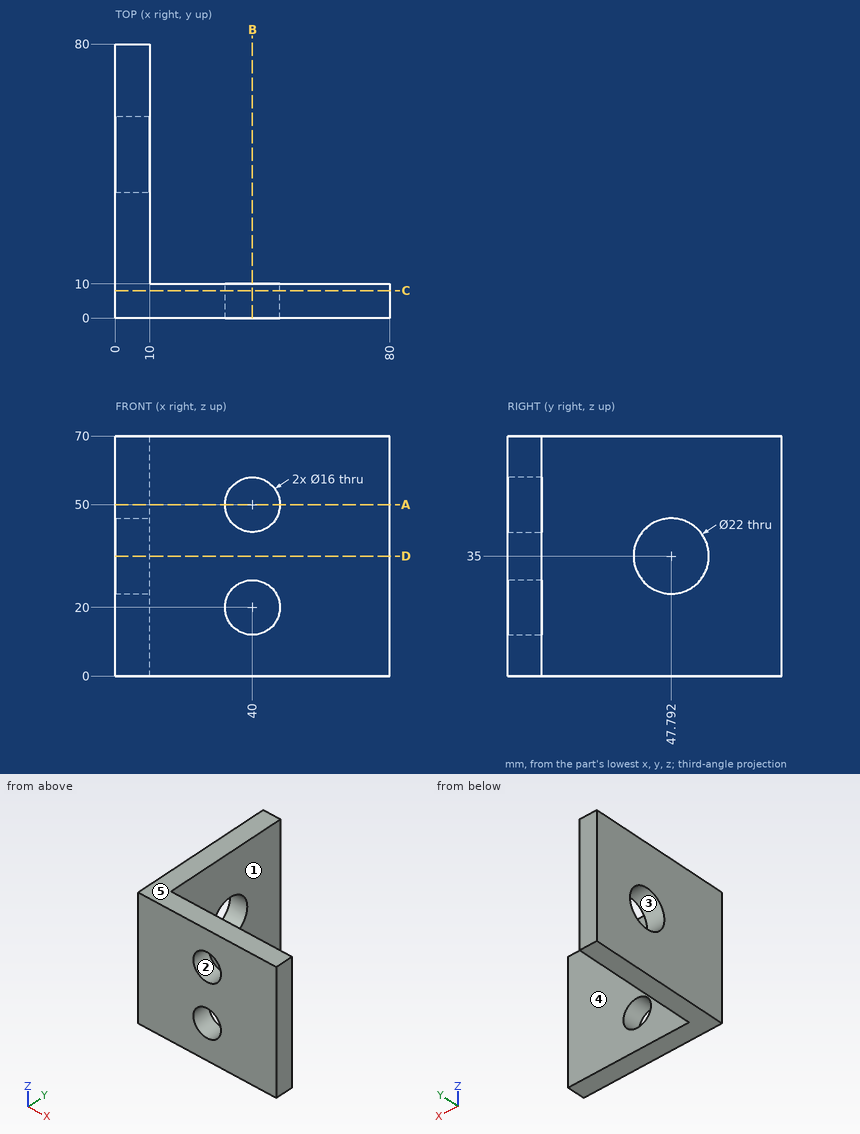
Design review of the part shown in the three views and the two pictorial views. Dimensions are in mm from the part's minimum x, y and z. A direction names the side the tool comes from. Give positions to 0.01 mm unless a question says otherwise; leave off trailing zeros. Loops run counter-clockwise (first coordinate to the right, second up) from the corner with the lowest first, then second, coordinate; pieces in that order, holes last. Notation, with made-up numbers: (-7, -35.5) -> (33, -35.5) arc R19 cw to (33, -28.5) -> close; hole circle Ø3 at (72, 53.25). An arc over 180 degrees is marked (long way). Put each result on its own line as item: value. Start each with the question number.
1. We need section B-B on x = 40. State the section outline as (y, z) points, then the cut area to 3 significant figures.
2. Wall thickness on probe 1 along X at (y, z) = (5.5, 50); probe 2 along Y at (x, z) = (13.5, 52): over which ranges is each line inside the solid? List them lowest first.
3. For the marked faces 4 and 5, list the 3-axis set-ups (+Z, -Z, +X, -X, +Y, -Y) from which the entire face can be reached by the end or side of a thin tool; tool diameter is ignored.
4. Clearance check with flat-ended pins moving along their axes: P1, Ø6, axis at x = 41.5, z = 9.5, coming from the -Y side; P2, Ø10, axis at y = 33, z = 47.5, coming from the +X side; P3, Ø18.5, axis at x = 40, z = 50, coming from the +Y side. State where each tip first meets the part, or that it passes through.
5. Mouldability with a two-part tool opening along X and no side actions: class the marked faces 1, 2 and 3 as released by +X, released by -X, zero draft, split by the parting line, or undercut.
6. We need section C-C on y = 8. State the section outline as (x, z) points.
7. We need section D-D on z = 35. State the section outline as (x, y) points, then the cut area to 3 significant figures.
8. We need section A-A on z = 50. State the section outline as (x, y) points.
Determined:
1. outline: (0, 0) -> (10, 0) -> (10, 12) -> (0, 12) -> close; (0, 28) -> (10, 28) -> (10, 42) -> (0, 42) -> close; (0, 58) -> (10, 58) -> (10, 70) -> (0, 70) -> close
1. area: 380 mm^2
2. probe 1: 0 to 32, 48 to 80
2. probe 2: 0 to 10
3. face 4: +Z, -Z, +X, +Y
3. face 5: +Z, +X, -X, +Y, -Y
4. P1: y = 0
4. P2: x = 10
4. P3: y = 10
5. face 1: released by +X
5. face 2: undercut
5. face 3: zero draft
6. outline: (0, 0) -> (80, 0) -> (80, 70) -> (0, 70) -> close; hole circle Ø16 at (40, 20); hole circle Ø16 at (40, 50)
7. outline: (0, 0) -> (80, 0) -> (80, 10) -> (10, 10) -> (10, 36.79) -> (0, 36.79) -> close; (0, 58.79) -> (10, 58.79) -> (10, 80) -> (0, 80) -> close
7. area: 1,280 mm^2
8. outline: (0, 0) -> (32, 0) -> (32, 10) -> (10, 10) -> (10, 80) -> (0, 80) -> close; (48, 0) -> (80, 0) -> (80, 10) -> (48, 10) -> close
